Geometry check sheet. Reference: the model listing, model coordinates, mm. A direction names the side the tool comes from. Give positions to 0.01 mm unless a question says otherwise; leave off trailing zeros. Write each loop counter-clockwise with the first axis right and the second up, starting at its lowest first coordinate (ties: lowest second). Pieces come first, ordered by that corner, then holes.
(1) Cross-section at B-B (z = 0). Record the boundary of the cut face in (x, y).
(2) Tool access check on faces 1 (the flat face through (70, 12, 1)), 2 (the flat face through (22, 647, 22)). Record the directions out of +Z, -Z, +X, -X, +Y, -Y that give a thin tool (end or side, any length) a straight path to the whole face; none if there is none.
(3) Depth check by flat-ended pin: P1, Ø1, axis at x = 33, y = 95, coming from the -Z side; P2, Ø20.5, axis at x = 55.5, z = -55.5, coming from the +Y side; P3, Ø1.5, axis at x = 13.5, y = 486.5, coming from the -Z side; P4, Ø12, axis at x = -54.5, z = -45.5, coming from the -Y side. Enter the tip coordinate at first touch or a pass-through.
(4) Thickness scan on line 1 along X through (y, z) = (18, 55); line 2 along X through (y, z) = (461, 0); line 3 along Y through (x, z) = (16, 61). Record the ranges inside material, lowest first.
(5) Mould release check, pull along Z, two halves, no side actions. Record for faces 3 (the cylindrical face through (15.02, 633.94, 47.69)), 4 (the cylindrical face through (58.203, 12.325, -46.916)), 5 (the flat face through (-1, 12, 70)), 6 (the flat face through (17, 0, -17)): +Z half, -Z half, draft (parallel to the pull), parting line (faces both ways), or undercut.
(6) Cross-section at A-A (x = 0). Record the boundary of the cut face in (y, z), and give its area (3 significant figures).
(7) Cross-section at C-C (y = 304). Record the boundary of the cut face in (x, z), and give its area (3 significant figures).
(8) Cross-section at D-D (z = -39). Record the boundary of the cut face in (x, y).
```python
from build123d import *

# Parameters (mm, degrees)
SKETCH1_W           = 140
SKETCH1_H           = 140
SKETCH1_R           = 9
BOSS_EXTRUDE1_DEPTH = 25
SKETCH2_R           = 55
BOSS_EXTRUDE2_DEPTH = 652
SKETCH3_R           = 20
CUT_EXTRUDE1_DEPTH  = 1580
SKETCH4_OUTSIDE_W   = 278.28
SKETCH4_OUTSIDE_H   = 278.28
SKETCH4_OUTSIDE_R   = 30
CUT_EXTRUDE2_DEPTH  = 5
SKETCH6_OUTSIDE_W   = 278.28
SKETCH6_OUTSIDE_H   = 278.28
SKETCH6_OUTSIDE_R   = 50
CUT_EXTRUDE3_DEPTH  = 31.5


with BuildPart() as part:
    # Sketch1 → Boss-Extrude1 (new body)
    with BuildSketch(Plane(origin=(0, 0, 0), x_dir=(1, 0, 0), z_dir=(0, 1, 0))):
        Rectangle(SKETCH1_W, SKETCH1_H)
        with Locations(Location((-55.5, 55.5, 0), (0, 0, 270))):
            Circle(SKETCH1_R, mode=Mode.SUBTRACT)
        with Locations(Location((55.5, 55.5, 0), (0, 0, 270))):
            Circle(SKETCH1_R, mode=Mode.SUBTRACT)
        with Locations(Location((55.5, -55.5, 0), (0, 0, 270))):
            Circle(SKETCH1_R, mode=Mode.SUBTRACT)
        with Locations(Location((-55.5, -55.5, 0), (0, 0, 270))):
            Circle(SKETCH1_R, mode=Mode.SUBTRACT)
    extrude(amount=BOSS_EXTRUDE1_DEPTH)

    # Sketch2 → Boss-Extrude2 (add)
    with BuildSketch(Plane(origin=(0, 0, 0), x_dir=(1, 0, 0), z_dir=(0, 1, 0))):
        with Locations(Location((0, 0, 0), (0, 0, 270))):
            Circle(SKETCH2_R)
    extrude(amount=BOSS_EXTRUDE2_DEPTH)

    # Sketch3 → Cut-Extrude1 (cut)
    with BuildSketch(Plane(origin=(0, 652, 0), x_dir=(1, 0, 0), z_dir=(0, 1, 0))):
        with Locations(Location((0, 0, 0), (0, 0, 270))):
            Circle(SKETCH3_R)
    extrude(amount=-CUT_EXTRUDE1_DEPTH, mode=Mode.SUBTRACT)

    # Sketch4 outside → Cut-Extrude2 (cut)
    with BuildSketch(Plane(origin=(0, 652, 0), x_dir=(1, 0, 0), z_dir=(0, 1, 0))):
        Rectangle(SKETCH4_OUTSIDE_W, SKETCH4_OUTSIDE_H)
        with Locations(Location((0, 0, 0), (0, 0, 270))):
            Circle(SKETCH4_OUTSIDE_R, mode=Mode.SUBTRACT)
    extrude(amount=-CUT_EXTRUDE2_DEPTH, mode=Mode.SUBTRACT)

    # Sketch6 outside → Cut-Extrude3 (cut)
    with BuildSketch(Plane(origin=(0, 652, 0), x_dir=(1, 0, 0), z_dir=(0, 1, 0))):
        Rectangle(SKETCH6_OUTSIDE_W, SKETCH6_OUTSIDE_H)
        with Locations(Location((0, 0, 0), (0, 0, 270))):
            Circle(SKETCH6_OUTSIDE_R, mode=Mode.SUBTRACT)
    extrude(amount=-CUT_EXTRUDE3_DEPTH, mode=Mode.SUBTRACT)


solid = part.part
```
Reply:
1. outline: (-70, 0) - (-20, 0) - (-20, 652) - (-30, 652) - (-30, 647) - (-50, 647) - (-50, 620.5) - (-55, 620.5) - (-55, 25) - (-70, 25) - close; (20, 0) - (70, 0) - (70, 25) - (55, 25) - (55, 620.5) - (50, 620.5) - (50, 647) - (30, 647) - (30, 652) - (20, 652) - close
2. face 1: +Z, -Z, +X, +Y, -Y
2. face 2: +Y
3. P1: stops at z = -44.37
3. P2: stops at y = 25
3. P3: stops at z = -53.5
3. P4: stops at y = 0
4. line 1: x = -70 to -64.49, -46.51 to 46.51, 64.49 to 70
4. line 2: x = -55 to -20, 20 to 55
4. line 3: y = 0 to 25
5. face 3: parting line
5. face 4: undercut
5. face 5: +Z half
5. face 6: draft
6. outline: (0, -70) - (25, -70) - (25, -55) - (620.5, -55) - (620.5, -50) - (647, -50) - (647, -30) - (652, -30) - (652, -20) - (0, -20) - close; (0, 20) - (652, 20) - (652, 30) - (647, 30) - (647, 50) - (620.5, 50) - (620.5, 55) - (25, 55) - (25, 70) - (0, 70) - close
6. area: 45,900 mm2
7. outline: circle Ø110 at (0, 0); hole circle Ø40 at (0, 0)
7. area: 8,250 mm2
8. outline: (-70, 0) - (70, 0) - (70, 25) - (38.78, 25) - (38.78, 620.5) - (31.29, 620.5) - (31.29, 647) - (-31.29, 647) - (-31.29, 620.5) - (-38.78, 620.5) - (-38.78, 25) - (-70, 25) - close
